Source: CAD feature listing. Evaluate the final solid. Frame: model axes, mm. Give positions to 0.01 mm unless a question says otherwise; leave off trailing zeros. Order: outer loops, then holes, each group sorted by start corner. A loop starts at its lowest first (then second) coordinate and runs counter-clockwise, first axis right, second up.
1) Draft query along X for faces 1 (the face through (-16, 4, -10)), 2 (the face through (-472.19, -0.06, -212.2)). Return one class per face: released by +X, released by -X, zero draft, split by the parting line, or undercut.
2) Section A-A, the plane x = -480. Return loops of the section in (y, z).
3) Section B-B, the plane z = -237. Return loops of the section in (x, y), plus the area to 3 significant figures.
4) Material intervals for line 1 (X direction, y = -2, z = -237), sorted ascending.
```python
from build123d import *

# Parameters (mm, degrees)
SKETCH_1_W      = 2324
SKETCH_1_H      = 1380
SKETCH_1_R      = 26
EXTRUDE_1_DEPTH = 4


with BuildPart() as part:
    # 草图1 → 凸台-拉伸1 (new, symmetric)
    with BuildSketch(Plane(origin=(0, 0, 0), x_dir=(1, 0, 0), z_dir=(0, 1, 0))):
        Rectangle(SKETCH_1_W, SKETCH_1_H)
        with Locations(Location((-480, 237, 0), (0, 0, 270))):
            Circle(SKETCH_1_R, mode=Mode.SUBTRACT)
    extrude(amount=EXTRUDE_1_DEPTH, both=True)


solid = part.part
```
From the geometry:
1. face 1: zero draft
1. face 2: undercut
2. outline: (-4, -690) - (4, -690) - (4, -263) - (-4, -263) - close; (-4, -211) - (4, -211) - (4, 690) - (-4, 690) - close
3. outline: (-1162, -4) - (-506, -4) - (-506, 4) - (-1162, 4) - close; (-454, -4) - (1162, -4) - (1162, 4) - (-454, 4) - close
3. area: 18,200 mm2
4. line 1: x = -1162 to -506, -454 to 1162
